Input: part model. Units: mm. Frame: model coordinates. Face numbers are marked on the shaded views. A direction names the side the tool comes from. Round coordinates to 2 decimals unless told otherwise and drop trailing zeros. Loops run counter-clockwise (first coordinate to the right, second up) from the corner with the lowest first, then second, coordinate; pieces in that order, holes last.
1) Section C-C, the plane z = 50.5. Return loops of the section in (x, y), and give its area (3 significant figures).
2) Draft query along Y for the marked faces 1, 2 and 3. Return one class per face: pulls with the +Y half, pulls with the -Y half, needs draft (parallel to the pull), parting line crosses it, or undercut.
3) Ray query, line 1 along X through (y, z) = (0, 8.95); line 2 along Y through (x, z) = (-146.75, 30); line 3 along Z through (x, y) = (1.5, -80). Return the intervals inside material, ascending.
4) Section B-B, the plane y = 75. Return loops of the section in (x, z).
5) First-contact query: pin 1 (6 mm diameter, centred on x = -5, y = -61.5, fed in from +Z); pin 2 (4 mm diameter, centred on y = -30.5, z = 52, fed in from -X); pin 3 (5 mm diameter, centred on y = -7.5, z = 20, fed in from -X). Flat tips, straight axial feed; report the tip coordinate or a pass-through.
6) Section D-D, the plane x = -44. Return loops of the section in (y, z), and give its area (3 significant figures).
7) Access query for the marked faces 4, 5, 6 and 7. Directions: +Z, -Z, +X, -X, +Y, -Y. A direction counts if a zero-diameter tool reaches every point of the face in a straight line with its end or side. Return the directions, or none.
8) Section A-A, the plane z = 30. Return loops of the section in (x, y).
from build123d import *

# Parameters (mm, degrees)
SKETCH_1_R          = 8
EXTRUDE_1_DEPTH     = 10
EXTRUDE_2_DEPTH     = 50
CUT_EXTRUDE_1_DEPTH = 188.082869339
SKETCH_4_R          = 10
CUT_EXTRUDE_2_DEPTH = 40
SKETCH_6_R          = 12
CUT_EXTRUDE_4_DEPTH = 5


with BuildPart() as part:
    # 草图1 → 凸台-拉伸1 (new body)
    with BuildSketch(Plane.XY):
        with BuildLine():
            Line((0, 100), (-150, 100))
            Line((-150, 100), (-150, -100))
            Line((-150, -100), (0, -100))
            ThreePointArc((0, -100), (100, 0), (0, 100))
        make_face()
        Circle(SKETCH_1_R, mode=Mode.SUBTRACT)
    extrude(amount=EXTRUDE_1_DEPTH)

    # 草图2 → 凸台-拉伸2 (add)
    with BuildSketch(Plane.XY.offset(10)):
        Polygon((-150, 42.426406871), (-150, 100), (-140, 100), (-140, 46.568542495), (-93.431457505, 0), (-140, -46.568542495), (-140, -100), (-150, -100), (-150, -42.426406871), (-107.573593129, 0), align=None)
    extrude(amount=EXTRUDE_2_DEPTH)

    # 草图3 → 切除-拉伸1 (cut, through all)
    with BuildSketch(Plane.XY.offset(10)):
        Polygon((-150, -42.426406871), (-107.573593129, 0), (-150, 42.426406871), align=None)
    extrude(amount=-CUT_EXTRUDE_1_DEPTH, mode=Mode.SUBTRACT)

    # 草图4 → 切除-拉伸2 (cut)
    with BuildSketch(Plane.ZY.offset(150)):
        with Locations((30, -75)):
            Circle(SKETCH_4_R)
        with Locations((30, 75)):
            Circle(SKETCH_4_R)
    extrude(amount=-CUT_EXTRUDE_2_DEPTH, mode=Mode.SUBTRACT)

    # 草图6 → 切除-拉伸4 (cut)
    with BuildSketch(Plane(origin=(0, 0, 0), x_dir=(-1, 0, 0), z_dir=(0, 0, -1))):
        Circle(SKETCH_6_R)
    extrude(amount=-CUT_EXTRUDE_4_DEPTH, mode=Mode.SUBTRACT)


solid = part.part
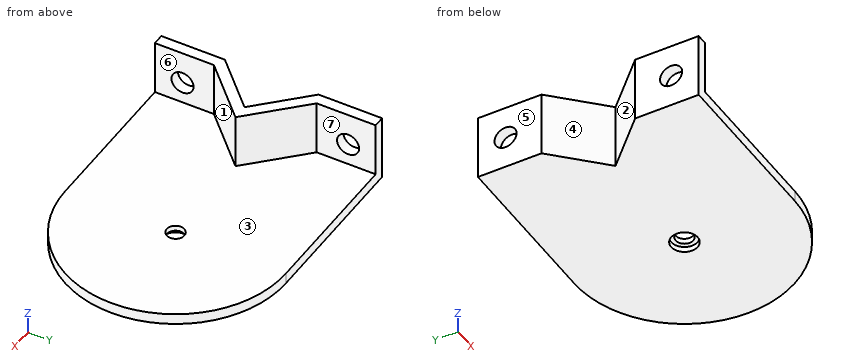
Final values:
1. outline: (-150, -100) - (-140, -100) - (-140, -46.57) - (-93.43, 0) - (-140, 46.57) - (-140, 100) - (-150, 100) - (-150, 42.43) - (-107.57, 0) - (-150, -42.43) - close
1. area: 2,370 mm2
2. face 1: pulls with the -Y half
2. face 2: undercut
2. face 3: needs draft
3. line 1: x = -107.57 to -8, 8 to 100
3. line 2: y = -100 to -85, -65 to -39.18, 39.18 to 65, 85 to 100
3. line 3: z = 0 to 10
4. outline: (-150, 0) - (66.14, 0) - (66.14, 10) - (-140, 10) - (-140, 20) - (-150, 20) - close; (-150, 40) - (-140, 40) - (-140, 60) - (-150, 60) - close
5. pin 1: stops at z = 10
5. pin 2: stops at x = -140.07
5. pin 3: stops at x = -117.57
6. outline: (-100, 0) - (100, 0) - (100, 10) - (-100, 10) - close
6. area: 2,000 mm2
7. face 4: +Z, -Z, -X
7. face 5: +Z, -Z, -X, +Y, -Y
7. face 6: +Z, +X, -Y
7. face 7: +Z, +X, +Y
8. outline: (-150, -100) - (-140, -100) - (-140, -85) - (-150, -85) - close; (-150, -65) - (-140, -65) - (-140, -46.57) - (-93.43, 0) - (-140, 46.57) - (-140, 65) - (-150, 65) - (-150, 42.43) - (-107.57, 0) - (-150, -42.43) - close; (-150, 85) - (-140, 85) - (-140, 100) - (-150, 100) - close
